Verification items for the finished model (mm, model axes). Give positions to 0.01 mm unless a question says otherwise; leave off trailing zeros. Order: outer loops, then holes, each group sorted by start corner. A loop starts at its lowest first (then second) coordinate and runs counter-clockwise, first axis right, second up. Notation, with made-up numbers: (74, 34.25) -> (133, 34.25) arc R22 cw to (133, 43.25) -> close; hole circle Ø9 at (63, 17). An arc over 180 degrees is marked (long way). Write each question's results on one line, items separated by ' | '. Start each with the question number.
1. Cross-section at C-C, the plane z = 43.5. Enter the section's corners in (x, y).
2. Cross-section at A-A, the plane x = -13. Enter the section's corners in (y, z).
3. Mould release check, pull along Y, two halves, no side actions. Record for faces 1 (the face through (-3, 362, 73.7)), 2 (the face through (3, 510, 69)), 3 (the face through (2.8, 240.551, 48.334)), 4 (the face through (-200, 362, 69)): +Y half, -Y half, draft (parallel to the pull), parting line (faces both ways), or undercut.
4. Cross-section at B-B, the plane y = 370. Enter the section's corners in (x, z), then the cut area to 3 significant figures.
5. Material ranges on L1, parallel to Z at x = -2, y = 422; L2, parallel to Z at x = -63, y = 254, recorded low to high. Write a range as from..to.
6. Depth check by flat-ended pin: pin 1 Ø10 at (x, z) = (14, 40.5) entering from -Y; pin 2 Ø2.5 at (x, y) = (50, 400) entering from +Z; pin 3 Ø2 at (x, y) = (-50, 300) entering from -Z. Enter the tip coordinate at first touch or a pass-through.
from build123d import *

# Parameters (mm, degrees)
EXTRUDE_1_DEPTH        = 200
EXTRUDE_1_DEPTH_BACK   = 200
SKETCH_6_W             = 360
SKETCH_6_H             = 260
CUT_EXTRUDE_1_DEPTH    = 3
CUT_EXTRUDE_2_REACH    = 370.623
HOLE_WIZARD_M4_1_D     = 3.3
HOLE_WIZARD_M4_1_DEPTH = 10.1
HOLE_WIZARD_M4_1_TIP   = 0.991420021


with BuildPart() as part:
    # 草图5 → 凸台-拉伸1 (new, two sides: drawn at the far end of the back side and taken through both)
    with BuildSketch(Plane.ZY.offset(-EXTRUDE_1_DEPTH_BACK)):
        Polygon((26.700089157, 410), (61.700089157, 510), (76.700089157, 510), (76.700089157, 210), (61.700089157, 210), (26.700089157, 290), align=None)
    extrude(amount=EXTRUDE_1_DEPTH + EXTRUDE_1_DEPTH_BACK)

    # 草图6 → 切除-拉伸1 (cut)
    with BuildSketch(Plane.XY.offset(76.700089157)):
        with Locations((0, 360)):
            Rectangle(SKETCH_6_W, SKETCH_6_H)
    extrude(amount=-CUT_EXTRUDE_1_DEPTH, mode=Mode.SUBTRACT)

    # 草图8 → 切除-拉伸2 (cut, up to next)
    with BuildSketch(Plane(origin=(0, 510, 0), x_dir=(1, 0, 0), z_dir=(0, 1, 0)), mode=Mode.PRIVATE) as cut_extrude_2_sk1:
        Polygon((-200, -61.700089157), (-200, -26.700089157), (-60, -26.700089157), align=None)
    cut_extrude_2_tool1 = extrude(cut_extrude_2_sk1.sketch, amount=-CUT_EXTRUDE_2_REACH, mode=Mode.PRIVATE) & part.part
    # 草图8 → 切除-拉伸2 (cut, up to next)
    with BuildSketch(Plane(origin=(0, 510, 0), x_dir=(1, 0, 0), z_dir=(0, 1, 0)), mode=Mode.PRIVATE) as cut_extrude_2_sk2:
        Polygon((60, -26.700089157), (200, -26.700089157), (200, -61.700089157), align=None)
    cut_extrude_2_tool2 = extrude(cut_extrude_2_sk2.sketch, amount=-CUT_EXTRUDE_2_REACH, mode=Mode.PRIVATE) & part.part
    add(cut_extrude_2_tool1.solids().sort_by_distance((-153.333333, 510, 38.366756))[0], mode=Mode.SUBTRACT)
    add(cut_extrude_2_tool2.solids().sort_by_distance((153.333333, 510, 38.366756))[0], mode=Mode.SUBTRACT)

    # M4 螺纹孔1
    with Locations(Plane(origin=(0, 0, 26.700089157), x_dir=(-1, 0, 0), z_dir=(0, 0, -1))):
        with Locations((-50, 400), (50, 400), (50, 300), (-50, 300)):
            Hole(HOLE_WIZARD_M4_1_D / 2, depth=HOLE_WIZARD_M4_1_DEPTH)
            with Locations((0, 0, -(HOLE_WIZARD_M4_1_DEPTH + HOLE_WIZARD_M4_1_TIP / 2))):  # 118° drill point
                Cone(0, HOLE_WIZARD_M4_1_D / 2, HOLE_WIZARD_M4_1_TIP, mode=Mode.SUBTRACT)


solid = part.part
Results below:
1) outline: (-127.2, 251.6) -> (127.2, 251.6) -> (127.2, 458) -> (-127.2, 458) -> close
2) outline: (210, 61.7) -> (290, 26.7) -> (410, 26.7) -> (510, 61.7) -> (510, 76.7) -> (490, 76.7) -> (490, 73.7) -> (230, 73.7) -> (230, 76.7) -> (210, 76.7) -> close
3) face 1: undercut | face 2: +Y half | face 3: -Y half | face 4: draft
4) outline: (-200, 61.7) -> (-60, 26.7) -> (60, 26.7) -> (200, 61.7) -> (200, 76.7) -> (180, 76.7) -> (180, 73.7) -> (-180, 73.7) -> (-180, 76.7) -> (-200, 76.7) -> close | area: 14,000 mm²
5) L1: z = 30.9..73.7 | L2: z = 42.45..73.7
6) pin 1: stops at y = 247.03 | pin 2: stops at z = 73.7 | pin 3: stops at z = 37.19
